Source: CAD feature listing. Evaluate the final solid. Frame: model axes, mm. Coordinates: 2 decimals unless noted, no trailing zeros. Write each loop counter-clockwise with the first axis right and the second up, starting at its lowest first coordinate (ties: lowest second). Pieces come first, ordered by that corner, then holes. Notation, with made-up numbers: (1.5, 78.5) - (30.5, 78.5) arc R23 ccw to (30.5, 110.5) - close; hole circle Ø7 at (14.25, 52.25). An arc over 180 degrees is marked (long way). One line per item, written item: value.
from build123d import *

# Parameters (mm, degrees)
SKETCH1_W           = 75
SKETCH1_H           = 20
SKETCH1_R           = 2
BOSS_EXTRUDE1_DEPTH = 5
FILLET1_R           = 5


with BuildPart() as part:
    # Sketch1 → Boss-Extrude1 (new body)
    with BuildSketch(Plane.XY):
        with Locations((37.5, -10)):
            Rectangle(SKETCH1_W, SKETCH1_H)
        with Locations((10, -10)):
            Circle(SKETCH1_R, mode=Mode.SUBTRACT)
        with Locations((65, -10)):
            Circle(SKETCH1_R, mode=Mode.SUBTRACT)
        with Locations((37.5, -10)):
            Circle(SKETCH1_R, mode=Mode.SUBTRACT)
    extrude(amount=BOSS_EXTRUDE1_DEPTH)

    # Fillet1
    fillet1_edges = [part.edges().sort_by_distance(p)[0] for p in [
        (0, 0, 2.5),
        (75, 0, 2.5),
    ]]
    fillet(fillet1_edges, radius=FILLET1_R)


solid = part.part
1) Draft query along X for faces 1 (the cylindrical face through (63.526, -8.648, 2.465)), 2 (the flat face through (37, 0, 2)), 3 (the cylindrical face through (73, -1, 3)), 4 (the flat face through (0, -13, 2)). Return one class per face: released by +X, released by -X, zero draft, split by the parting line, or undercut.
Values found:
face 1: undercut
face 2: zero draft
face 3: released by +X
face 4: released by -X
2) Section query C-C on x = 65. Output: boundary loops of the cut face in (y, z), then the cut area to 3 significant figures.
Values found:
outline: (-20, 0) - (-12, 0) - (-12, 5) - (-20, 5) - close; (-8, 0) - (0, 0) - (0, 5) - (-8, 5) - close
area: 80.0 mm2
3) Section query A-A on y = -10. Output: boundary loops of the cut face in (x, z), then the cut area to 3 significant figures.
Values found:
outline: (0, 0) - (8, 0) - (8, 5) - (0, 5) - close; (12, 0) - (35.5, 0) - (35.5, 5) - (12, 5) - close; (39.5, 0) - (63, 0) - (63, 5) - (39.5, 5) - close; (67, 0) - (75, 0) - (75, 5) - (67, 5) - close
area: 315 mm2
4) Section query D-D on y = -1.5. Output: boundary loops of the cut face in (x, z).
Values found:
outline: (1.43, 0) - (73.57, 0) - (73.57, 5) - (1.43, 5) - close
5) Section query B-B on z = 4.25. Output: boundary loops of the cut face in (x, y), then the cut area to 3 significant figures.
Values found:
outline: (0, -20) - (75, -20) - (75, -5) arc R5 ccw to (70, 0) - (5, 0) arc R5 ccw to (0, -5) - close; hole circle Ø4 at (10, -10); hole circle Ø4 at (37.5, -10); hole circle Ø4 at (65, -10)
area: 1,450 mm2
6) Material intervals for line 1 (X direction, y = -10.25, z = 4); line 2 (Y direction, x = 10, z = 2.3); line 3 (X direction, y = -11.5, z = 2.6), sorted ascending.
Values found:
line 1: 0 to 8.02, 11.98 to 35.52, 39.48 to 63.02, 66.98 to 75
line 2: -20 to -12, -8 to 0
line 3: 0 to 8.68, 11.32 to 36.18, 38.82 to 63.68, 66.32 to 75
7) Contact query for a flat-ended pin moving along its axis: P1, Ø5, axis at x = 10, y = -10, coming from the +Z side. Output: stop coordinate, or through.
Values found:
P1: z = 5
